Geometry check sheet. Reference: the model listing, model coordinates, mm. Face numbers are marked on the shaded views. A direction names the side the tool comes from. Give positions to 0.01 mm unless a question says otherwise; leave off trailing zeros. Loops run counter-clockwise (first coordinate to the right, second up) from the corner with the lowest first, then second, coordinate; pieces in that order, holes last. Notation, with made-up numbers: (-8, 35.25) -> (30, 35.25) arc R23 ccw to (30, 46.25) -> close; hole circle Ø7 at (32.25, -36.75). An arc over 180 degrees is marked (long way). Write item = value, one per line. Start each with the question number.
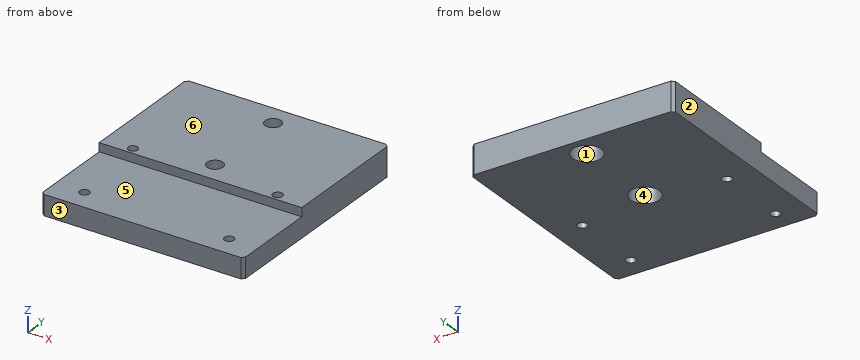
```python
from build123d import *

# Parameters (mm, degrees)
SKETCH1_W                                            = 70
SKETCH1_H                                            = 75
BOSS_EXTRUDE1_DEPTH                                  = 10
SKETCH2_W                                            = 3
SKETCH2_H                                            = 30
CUT_EXTRUDE1_DEPTH                                   = 104.07764064
M4_TAPPED_HOLE1_D                                    = 3.3
M4_TAPPED_HOLE1_DEPTH                                = 11.5
M4_TAPPED_HOLE1_TIP                                  = 0.991420021
HOLE_SIZE_PER_SOCKET_HEAD_CAP_SCREW_TYPE_D           = 5.5
HOLE_SIZE_PER_SOCKET_HEAD_CAP_SCREW_TYPE_CBORE_D     = 10
HOLE_SIZE_PER_SOCKET_HEAD_CAP_SCREW_TYPE_CBORE_DEPTH = 5.7
CHAMFER1_SIZE                                        = 1


with BuildPart() as part:
    # Sketch1 → Boss-Extrude1 (new body)
    with BuildSketch(Plane.XY):
        with Locations((35, 37.5)):
            Rectangle(SKETCH1_W, SKETCH1_H)
    extrude(amount=BOSS_EXTRUDE1_DEPTH)

    # Sketch2 → Cut-Extrude1 (cut, through all)
    with BuildSketch(Plane.ZY):
        with Locations((8.5, 15)):
            Rectangle(SKETCH2_W, SKETCH2_H)
    extrude(amount=-CUT_EXTRUDE1_DEPTH, mode=Mode.SUBTRACT)

    # M4 Tapped Hole1
    with Locations(Plane(origin=(0, 0, 0), x_dir=(-1, 0, 0), z_dir=(0, 0, -1))):
        with Locations((-10, 7.5), (-10, 32.5), (-60, 7.5), (-60, 32.5)):
            Hole(M4_TAPPED_HOLE1_D / 2, depth=M4_TAPPED_HOLE1_DEPTH)
            with Locations((0, 0, -(M4_TAPPED_HOLE1_DEPTH + M4_TAPPED_HOLE1_TIP / 2))):  # 118° drill point
                Cone(0, M4_TAPPED_HOLE1_D / 2, M4_TAPPED_HOLE1_TIP, mode=Mode.SUBTRACT)

    # Hole Size per Socket Head Cap Screw Type0 (through all)
    with Locations(Plane(origin=(0, 0, 0), x_dir=(-1, 0, 0), z_dir=(0, 0, -1))):
        with Locations((-35, 37.5), (-35, 67.5)):
            CounterBoreHole(HOLE_SIZE_PER_SOCKET_HEAD_CAP_SCREW_TYPE_D / 2, HOLE_SIZE_PER_SOCKET_HEAD_CAP_SCREW_TYPE_CBORE_D / 2, HOLE_SIZE_PER_SOCKET_HEAD_CAP_SCREW_TYPE_CBORE_DEPTH)

    # Chamfer1
    chamfer1_edges = [part.edges().sort_by_distance(p)[0] for p in [
        (70, 0, 3.5),
        (0, 0, 3.5),
        (0, 75, 5),
        (70, 75, 5),
    ]]
    chamfer(chamfer1_edges, length=CHAMFER1_SIZE)


solid = part.part
```
1) Section check A-A (y = 7.5). Enter the section's corners in (x, z), plus the area to 3 significant figures.
2) Thickness scan on line 1 (Y direction, x = 35, z = 6.8); line 2 (Y direction, x = 35, z = 8.75); line 3 (Y direction, x = 60, z = 9.5). Record the ranges inside material, lowest first.
3) Depth check by flat-ended pin: pin 1 Ø9 at (x, y) = (45, 9.5) entering from +Z; pin 2 Ø2.5 at (x, z) = (44, 9) entering from -Y; pin 3 Ø6.5 at (x, y) = (35, 37.5) entering from -Z. Enter the tip coordinate at first touch or a pass-through.
4) Section check B-B (x = 10). Enter the section's corners in (y, z), plus the area to 3 significant figures.
5) Section check D-D (x = 35). Enter the section's corners in (y, z), plus the area to 3 significant figures.
6) Section check C-C (z = 2). Enter the section's corners in (x, y).
7) Tool access check on the marked faces 4, 5 and 6. Record the directions out of +Z, -Z, +X, -X, +Y, -Y that give a thin tool (end or side, any length) a straight path to the whole face; none if there is none.
8) Draft check along Y on the marked faces 1, 2 and 3. Enter one of: released by +Y, released by -Y, zero draft, split by the parting line, or undercut.
Check result:
q1.outline = (0, 0) -> (8.35, 0) -> (8.35, 7) -> (0, 7) -> close; (11.65, 0) -> (58.35, 0) -> (58.35, 7) -> (11.65, 7) -> close; (61.65, 0) -> (70, 0) -> (70, 7) -> (61.65, 7) -> close
q1.area = 444 mm2
q2.line_1 = 0 to 34.75, 40.25 to 64.75, 70.25 to 75
q2.line_2 = 30 to 34.75, 40.25 to 64.75, 70.25 to 75
q2.line_3 = 30 to 30.85, 34.15 to 75
q3.pin_1 = 7
q3.pin_2 = 30
q3.pin_3 = 5.7
q4.outline = (0, 0) -> (5.85, 0) -> (5.85, 7) -> (0, 7) -> close; (9.15, 0) -> (30.85, 0) -> (30.85, 10) -> (30, 10) -> (30, 7) -> (9.15, 7) -> close; (34.15, 0) -> (75, 0) -> (75, 10) -> (34.15, 10) -> close
q4.area = 604 mm2
q5.outline = (0, 0) -> (32.5, 0) -> (32.5, 5.7) -> (34.75, 5.7) -> (34.75, 10) -> (30, 10) -> (30, 7) -> (0, 7) -> close; (40.25, 5.7) -> (42.5, 5.7) -> (42.5, 0) -> (62.5, 0) -> (62.5, 5.7) -> (64.75, 5.7) -> (64.75, 10) -> (40.25, 10) -> close; (70.25, 5.7) -> (72.5, 5.7) -> (72.5, 0) -> (75, 0) -> (75, 10) -> (70.25, 10) -> close
q5.area = 499 mm2
q6.outline = (0, 1) -> (1, 0) -> (69, 0) -> (70, 1) -> (70, 74) -> (69, 75) -> (1, 75) -> (0, 74) -> close; hole circle Ø3.3 at (10, 7.5); hole circle Ø3.3 at (10, 32.5); hole circle Ø10 at (35, 37.5); hole circle Ø10 at (35, 67.5); hole circle Ø3.3 at (60, 7.5); hole circle Ø3.3 at (60, 32.5)
q7.face_4 = -Z
q7.face_5 = +Z, +X, -X, -Y
q7.face_6 = +Z, +X, -X, +Y, -Y
q8.face_1 = undercut
q8.face_2 = zero draft
q8.face_3 = released by -Y
